```python
from build123d import *

# Parameters (mm, degrees)
SKETCH1_W                                            = 91
SKETCH1_H                                            = 28
BOSS_EXTRUDE1_DEPTH                                  = 7
M6_TAPPED_HOLE1_D                                    = 5
M6_TAPPED_HOLE1_DEPTH                                = 15
M6_TAPPED_HOLE1_TIP                                  = 1.502151548
HOLE_SIZE_PER_SOCKET_HEAD_CAP_SCREW_TYPE_D           = 5.5
HOLE_SIZE_PER_SOCKET_HEAD_CAP_SCREW_TYPE_CBORE_D     = 10
HOLE_SIZE_PER_SOCKET_HEAD_CAP_SCREW_TYPE_CBORE_DEPTH = 10
CHAMFER1_SIZE                                        = 1


with BuildPart() as part:
    # Sketch1 → Boss-Extrude1 (new, symmetric)
    with BuildSketch(Plane.XY):
        Rectangle(SKETCH1_W, SKETCH1_H)
    extrude(amount=BOSS_EXTRUDE1_DEPTH, both=True)

    # M6 Tapped Hole1
    with Locations(Plane.ZY.offset(45.5)):
        with Locations((0, -7), (0, 7)):
            Hole(M6_TAPPED_HOLE1_D / 2, depth=M6_TAPPED_HOLE1_DEPTH)
            with Locations((0, 0, -(M6_TAPPED_HOLE1_DEPTH + M6_TAPPED_HOLE1_TIP / 2))):  # 118° drill point
                Cone(0, M6_TAPPED_HOLE1_D / 2, M6_TAPPED_HOLE1_TIP, mode=Mode.SUBTRACT)

    # Hole Size per Socket Head Cap Screw Type1 (through all)
    with Locations(Plane(origin=(0, 14, 0), x_dir=(1, 0, 0), z_dir=(0, 1, 0))):
        with Locations((7.5, 0), (-20.5, 0), (35.5, 0)):
            CounterBoreHole(HOLE_SIZE_PER_SOCKET_HEAD_CAP_SCREW_TYPE_D / 2, HOLE_SIZE_PER_SOCKET_HEAD_CAP_SCREW_TYPE_CBORE_D / 2, HOLE_SIZE_PER_SOCKET_HEAD_CAP_SCREW_TYPE_CBORE_DEPTH)

    # Chamfer1
    chamfer1_edges = [part.edges().sort_by_distance(p)[0] for p in [
        (45.5, -14, 0),
        (-45.5, -14, 0),
        (-45.5, 14, 0),
        (45.5, 14, 0),
    ]]
    chamfer(chamfer1_edges, length=CHAMFER1_SIZE)


solid = part.part
```
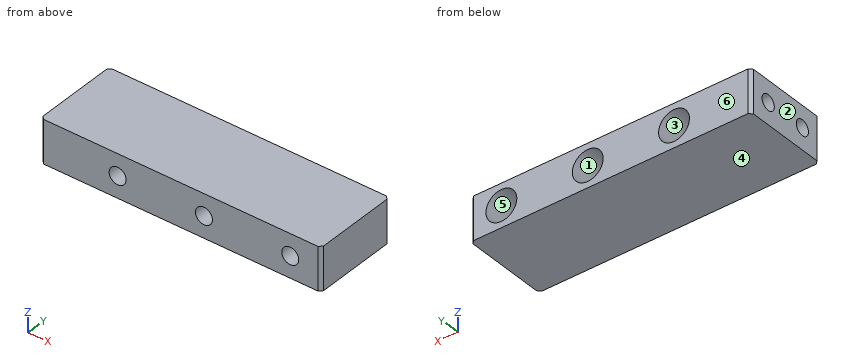
Work out the finished part from the listing and answer in its coordinate system (mm). Face numbers are marked on the shaded views. A direction names the side the tool comes from. Give positions to 0.01 mm unless a question says otherwise; leave off trailing zeros. Write each loop counter-clockwise with the first axis right and the second up, starting at its lowest first coordinate (ties: lowest second). Pieces come first, ordered by that corner, then holes.
(1) The part is cut by section A-A on x = 7.5. Write down the section's boundary in (y, z).
Final values:
outline: (-14, -7) - (14, -7) - (14, -5) - (4, -5) - (4, -2.75) - (-14, -2.75) - close; (-14, 2.75) - (4, 2.75) - (4, 5) - (14, 5) - (14, 7) - (-14, 7) - close
(2) The part is cut by section B-B on y = 2. Write down the section's boundary in (x, z), plus the area to 3 significant figures.
Final values:
outline: (-45.5, -7) - (45.5, -7) - (45.5, 7) - (-45.5, 7) - close; hole circle Ø5.5 at (-20.5, 0); hole circle Ø5.5 at (7.5, 0); hole circle Ø5.5 at (35.5, 0)
area: 1,200 mm2
(3) Straight lines are drawn through the part: line 1 (Y direction, x = -41.75, z = 0); line 2 (Z direction, x = -35.75, y = -7); line 3 (Z direction, x = 7.5, y = 8.5). For each, find the intervals that lie inside material, in ascending order.
Final values:
line 1: y = -14 to -9.5, -4.5 to 4.5, 9.5 to 14
line 2: z = -7 to -2.5, 2.5 to 7
line 3: z = -7 to -5, 5 to 7
(4) The part is cut by section C-C on x = -38. Write down the section's boundary in (y, z).
Final values:
outline: (-14, -7) - (14, -7) - (14, 7) - (-14, 7) - close; hole circle Ø5 at (-7, 0); hole circle Ø5 at (7, 0)
(5) A flat-ended cylindrical pin translates along its axis: pin 1 Ø1.5 at (x, z) = (32, 0) entering from +Y. Find the tip coordinate at first contact, or state that the pin passes through.
Final values:
pin 1: stops at y = 4
(6) The mould has two halves that part along X. Classify the marked faces 1, 2, 3 and 4: pulls with the +X half, pulls with the -X half, needs draft (parallel to the pull), parting line crosses it, or undercut.
Final values:
face 1: undercut
face 2: pulls with the -X half
face 3: undercut
face 4: needs draft
(7) Which of the six approach directions +Z, -Z, +X, -X, +Y, -Y give full straight-line access (tool end or side, diameter ignored) to the marked faces 5 and 6?
Final values:
face 5: +Y
face 6: +Z, -Z, +X, -X, +Y
